from build123d import *

# Parameters (mm, degrees)
SKETCH_1_W              = 310
SKETCH_1_H              = 310
EXTRUDE_1_DEPTH         = 20
FILLET_1_R              = 20
CUT_EXTRUDE_1_DEPTH     = 10
HOLE_WIZARD_M12_1_D     = 10.2
HOLE_WIZARD_M12_1_DEPTH = 15
HOLE_WIZARD_M12_1_TIP   = 3.064389157
CHAMFER_1_SIZE          = 5


with BuildPart() as part:
    # 草图1 → 凸台-拉伸1 (new body)
    with BuildSketch(Plane.XY):
        Rectangle(SKETCH_1_W, SKETCH_1_H)
        with BuildLine():
            Line((-94, 112), (94, 112))
            ThreePointArc((94, 112), (106.727922061, 106.727922061), (112, 94))
            Line((112, 94), (112, -94))
            ThreePointArc((112, -94), (106.727922061, -106.727922061), (94, -112))
            Line((94, -112), (-94, -112))
            ThreePointArc((-94, -112), (-106.727922061, -106.727922061), (-112, -94))
            Line((-112, -94), (-112, 94))
            ThreePointArc((-112, 94), (-106.727922061, 106.727922061), (-94, 112))
        make_face(mode=Mode.SUBTRACT)
    extrude(amount=EXTRUDE_1_DEPTH)

    # 圆角1
    fillet_1_edges = [part.edges().sort_by_distance(p)[0] for p in [
        (155, -155, 10),
        (-155, -155, 10),
        (-155, 155, 10),
        (155, 155, 10),
    ]]
    fillet(fillet_1_edges, radius=FILLET_1_R)

    # 草图2 → 切除-拉伸1 (cut)
    with BuildSketch(Plane(origin=(0, 0, 0), x_dir=(-1, 0, 0), z_dir=(0, 0, -1))):
        with BuildLine():
            Line((125.1, -95.1), (125.1, 95.1))
            ThreePointArc((125.1, 95.1), (116.313203436, 116.313203436), (95.1, 125.1))
            Line((95.1, 125.1), (-95.1, 125.1))
            ThreePointArc((-95.1, 125.1), (-116.313203436, 116.313203436), (-125.1, 95.1))
            Line((-125.1, 95.1), (-125.1, -95.1))
            ThreePointArc((-125.1, -95.1), (-116.313203436, -116.313203436), (-95.1, -125.1))
            Line((-95.1, -125.1), (95.1, -125.1))
            ThreePointArc((95.1, -125.1), (116.313203436, -116.313203436), (125.1, -95.1))
        make_face()
    extrude(amount=-CUT_EXTRUDE_1_DEPTH, mode=Mode.SUBTRACT)

    # M12 螺纹孔1
    with Locations(Plane(origin=(-137, 137, 20), x_dir=(1, 0, 0), z_dir=(0, 0, 1))):
        with Locations((0, 0), (274, 0), (274, -274), (0, -274), (137, -274), (137, 0), (0, -122), (0, -152), (274, -122), (274, -152)):
            Hole(HOLE_WIZARD_M12_1_D / 2, depth=HOLE_WIZARD_M12_1_DEPTH)
            with Locations((0, 0, -(HOLE_WIZARD_M12_1_DEPTH + HOLE_WIZARD_M12_1_TIP / 2))):  # 118° drill point
                Cone(0, HOLE_WIZARD_M12_1_D / 2, HOLE_WIZARD_M12_1_TIP, mode=Mode.SUBTRACT)

    # 倒角1
    chamfer_1_edges = [part.edges().sort_by_distance(p)[0] for p in [
        (106.727922061, -106.727922061, 20),
        (112, 0, 20),
        (106.727922061, 106.727922061, 20),
        (0, 112, 20),
        (-106.727922061, 106.727922061, 20),
        (-112, 0, 20),
        (-106.727922061, -106.727922061, 20),
        (0, -112, 20),
    ]]
    chamfer(chamfer_1_edges, length=CHAMFER_1_SIZE)


solid = part.part
The model under review builds one solid part; all positions refer to its coordinate system, in mm. A direction names the side the tool comes from. Give positions to 0.01 mm unless a question says otherwise; leave off trailing zeros. Loops run counter-clockwise (first coordinate to the right, second up) from the corner with the lowest first, then second, coordinate; pieces in that order, holes last. Notation, with made-up numbers: (-38.75, -37) -> (1.25, -37) arc R23 cw to (1.25, 0) -> close; hole circle Ø2 at (61, 60). An arc over 180 degrees is marked (long way). Answer as a JSON object with one key per item and string values. Group by question number.
Q1. Take a section at C-C (y = 121). Write out the cut boundary in (x, z).
Q2. Insertion check: pin 1 (1.5 mm diameter, centred on x = 20.5, y = 115, fed in from -Z); pin 2 (9 mm diameter, centred on x = 137, y = 137, fed in from +Z). Each pin has a flat end and moves straight along its axis. Give the tip position at first contact, or say it passes through.
Q3. Wall thickness on line 1 along Y through (x, z) = (89, 6.75); line 2 along Y through (x, z) = (-137, 8.5); line 3 along X through (y, z) = (-137, 11.75): over which ranges is each line inside the solid? List them lowest first.
Q4. Take a section at A-A (x = 54). Write out the cut boundary in (y, z), plus the area to 3 significant figures.
Q5. Tool access review of faces 5 (the conical face through (-107.83, 107.53, 16.35)), 6 (the cylindrical face through (106.587, 106.867, 12.465)), 7 (the cylindrical face through (148.986, 149.297, 10.14)): name each direction out of +Z, -Z, +X, -X, +Y, -Y from which nothing blocks a thin tool from reaching the whole face with its end or side.
Q6. Draft analysis for pull direction Y (two halves, no side actions). For faces 1 (the flat face through (-155, -2, 10)), 2 (the cylindrical face through (116.079, 116.545, 4.93)), 3 (the cylindrical face through (1, 132, 12)), 4 (the cylindrical face through (-149.297, 148.986, 10.14)), state which applies: pulls with the +Y half, pulls with the -Y half, needs draft (parallel to the pull), parting line crosses it, or undercut.
Answer below:
{
 "1": {"outline": "(-155, 0) -> (-110.24, 0) -> (-110.24, 10) -> (110.24, 10) -> (110.24, 0) -> (155, 0) -> (155, 20) -> (-155, 20) -> close"},
 "2": {"pin 1": "stops at z = 10", "pin 2": "stops at z = 4.64"},
 "3": {"line 1": "y = -155 to -125.1, 125.1 to 155", "line 2": "y = -154.9 to -142.1, -131.9 to -20.1, -9.9 to 9.9, 20.1 to 131.9, 142.1 to 154.9", "line 3": "x = -154.9 to -142.1, -131.9 to -5.1, 5.1 to 131.9, 142.1 to 154.9"},
 "4": {"outline": "(-155, 0) -> (-125.1, 0) -> (-125.1, 10) -> (-112, 10) -> (-112, 15) -> (-117, 20) -> (-155, 20) -> close; (112, 10) -> (125.1, 10) -> (125.1, 0) -> (155, 0) -> (155, 20) -> (117, 20) -> (112, 15) -> close", "area": "1,430 mm2"},
 "5": {"face 5": "+Z", "face 6": "+Z, -Z", "face 7": "+Z, -Z, +X, +Y"},
 "6": {"face 1": "needs draft", "face 2": "undercut", "face 3": "undercut", "face 4": "pulls with the +Y half"}
}
